```python
from build123d import *

# Parameters (mm, degrees)
SKETCH1_W             = 50
SKETCH1_H             = 50
BOSS_EXTRUDE1_DEPTH   = 35
SKETCH2_R             = 18
BOSS_EXTRUDE2_DEPTH   = 18
BOSS_EXTRUDE3_DEPTH   = 6
M6_TAPPED_HOLE1_D     = 5
M6_TAPPED_HOLE1_DEPTH = 17
M6_TAPPED_HOLE1_TIP   = 1.502151548


with BuildPart() as part:
    # Sketch1 → Boss-Extrude1 (new body)
    with BuildSketch(Plane(origin=(0, 0, 0), x_dir=(1, 0, 0), z_dir=(0, 1, 0))):
        Rectangle(SKETCH1_W, SKETCH1_H)
    extrude(amount=BOSS_EXTRUDE1_DEPTH)

    # Sketch2 → Boss-Extrude2 (add)
    with BuildSketch(Plane(origin=(0, 35, 0), x_dir=(1, 0, 0), z_dir=(0, 1, 0))):
        with Locations(Location((0, 0, 0), (0, 0, 270))):
            Circle(SKETCH2_R)
    extrude(amount=BOSS_EXTRUDE2_DEPTH)

    # Sketch3 → Boss-Extrude3 (add)
    with BuildSketch(Plane.XY.offset(25)):
        with BuildLine():
            Line((11.75, 32), (-11.75, 32))
            Line((-11.75, 32), (-11.75, 16.75))
            ThreePointArc((-11.75, 16.75), (0, 5), (11.75, 16.75))
            Line((11.75, 16.75), (11.75, 32))
        make_face()
    extrude(amount=BOSS_EXTRUDE3_DEPTH)

    # M6 Tapped Hole1
    with Locations(Plane.XY.offset(31)):
        with Locations((0, 16.75)):
            Hole(M6_TAPPED_HOLE1_D / 2, depth=M6_TAPPED_HOLE1_DEPTH)
            with Locations((0, 0, -(M6_TAPPED_HOLE1_DEPTH + M6_TAPPED_HOLE1_TIP / 2))):  # 118° drill point
                Cone(0, M6_TAPPED_HOLE1_D / 2, M6_TAPPED_HOLE1_TIP, mode=Mode.SUBTRACT)


solid = part.part
```
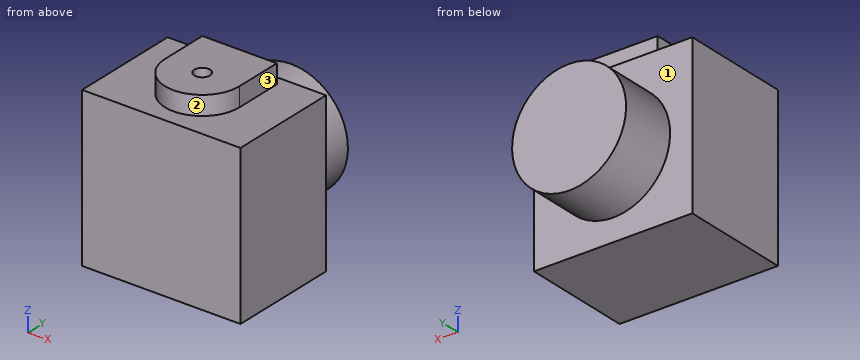
Can you work these out from the model? Positions are in its coordinate system, mm. Face numbers are marked on the shaded views. A direction names the side the tool comes from. Coordinates: 2 decimals unless noted, no trailing zeros. Order: outer loops, then holes, each group sorted by start corner. A loop starts at its lowest first (then second) coordinate and runs counter-clockwise, first axis right, second up.
1. For the marked faces 1, 2 and 3, which set-ups out of +Z, -Z, +X, -X, +Y, -Y let a thin tool reach every point of the face, with its end or its side?
2. If we section it at A-A (y = 28): Please give me the cut outline in (x, z).
3. I'm going to push flat-ended pins straight in: pin 1 (4 mm diameter, centred on x = 13, y = 43, fed in from -Z); pin 2 (8 mm diameter, centred on y = 42, z = 11, fed in from -X); pin 3 (4.5 mm diameter, centred on x = 0, y = 16.75, fed in from +Z). Where does each tip first touch, or does it pass through?
4. If we section it at C-C (x = -20.5): Please give me the cut outline in (y, z).
5. I need wall thicknesses on line 1 (Y direction, x = 0, z = 20); line 2 (X direction, y = 16.75, z = 24.75); line 3 (Y direction, x = 0, z = 26). Which ranges of each line are inside material? Lowest first, please.
6. If we section it at B-B (z = 0): Please give me the cut outline in (x, y).
7. If we section it at D-D (y = 37): Please give me the cut outline in (x, z).
Entries:
1. face 1: +Y
1. face 2: +Z, -Y
1. face 3: +Z, +X, +Y, -Y
2. outline: (-25, -25) - (25, -25) - (25, 25) - (11.75, 25) - (11.75, 31) - (-11.75, 31) - (-11.75, 25) - (-25, 25) - close
3. pin 1: stops at z = -14.25
3. pin 2: stops at x = -16.58
3. pin 3: stops at z = 13.85
4. outline: (0, -25) - (35, -25) - (35, 25) - (0, 25) - close
5. line 1: y = 0 to 14.25, 19.25 to 35
5. line 2: x = -25 to -2.5, 2.5 to 25
5. line 3: y = 5 to 14.25, 19.25 to 32
6. outline: (-25, 0) - (25, 0) - (25, 35) - (18, 35) - (18, 53) - (-18, 53) - (-18, 35) - (-25, 35) - close
7. outline: circle Ø36 at (0, 0)
